from build123d import *

# Parameters (mm, degrees)
SKETCH_1_R              = 67.5
SKETCH_1_R_2            = 32.5
EXTRUDE_1_DEPTH         = 3
HOLE_WIZARD_M12_1_D     = 10.2
HOLE_WIZARD_M12_1_DEPTH = 5
HOLE_WIZARD_M12_1_TIP   = 3.064389157


with BuildPart() as part:
    # 草图1 → 凸台-拉伸1 (new body)
    with BuildSketch(Plane(origin=(0, 0, 0), x_dir=(1, 0, 0), z_dir=(0, 1, 0))):
        with Locations(Location((0, 0, 0), (0, 0, 270))):
            Circle(SKETCH_1_R)
        with Locations(Location((0, 0, 0), (0, 0, 270))):
            Circle(SKETCH_1_R_2, mode=Mode.SUBTRACT)
    extrude(amount=EXTRUDE_1_DEPTH)

    # M12 螺纹孔的螺纹孔钻头1
    with Locations(Plane(origin=(0, 3, 0), x_dir=(1, 0, 0), z_dir=(0, 1, 0))):
        with Locations((0, 55), (-47.631397208, 27.5), (-47.631397208, -27.5), (0, -55), (47.631397208, -27.5), (47.631397208, 27.5)):
            Hole(HOLE_WIZARD_M12_1_D / 2, depth=HOLE_WIZARD_M12_1_DEPTH)
            with Locations((0, 0, -(HOLE_WIZARD_M12_1_DEPTH + HOLE_WIZARD_M12_1_TIP / 2))):  # 118° drill point
                Cone(0, HOLE_WIZARD_M12_1_D / 2, HOLE_WIZARD_M12_1_TIP, mode=Mode.SUBTRACT)


solid = part.part
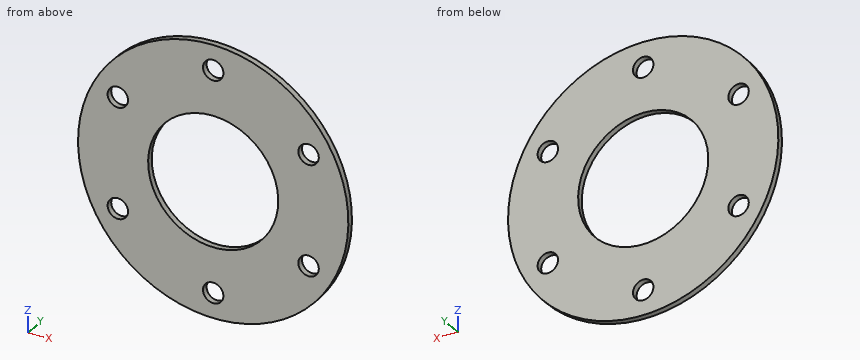
Input: part model. Units: mm. Frame: model coordinates. Coordinates: 2 decimals unless noted, no trailing zeros. Order: outer loops, then holes, each group sorted by start corner. A loop starts at its lowest first (then second) coordinate and runs counter-clockwise, first axis right, second up. Notation, with made-up numbers: M 81.5,-38 L 135.5,-38 A33 ccw 135.5,-9 Z; hole C 27.25,25 d1. An arc over 180 degrees is marked long. Answer in a Markdown table with one row per item.
(1) Material intervals for line 1 (Z direction, x = 52, y = 0.65); line 2 (X direction, y = 0.75, z = 0); line 3 (X direction, y = 1.45, z = -27.5), sorted ascending. Write a range as [from, to].
Numbers:
| item | result |
|---|---|
| line 1 | z = [-43.04, -30.13], [-24.87, 24.87], [30.13, 43.04] |
| line 2 | x = [-67.5, -32.5], [32.5, 67.5] |
| line 3 | x = [-61.64, -52.73], [-42.53, -17.32], [17.32, 42.53], [52.73, 61.64] |
(2) Section query C-C, the plane z = -27.5. Output: boundary loops of the cut face in (x, y).
Numbers:
| item | result |
|---|---|
| outline | M -61.64,0 L -52.73,0 L -52.73,3 L -61.64,3 Z; M -42.53,0 L -17.32,0 L -17.32,3 L -42.53,3 Z; M 17.32,0 L 42.53,0 L 42.53,3 L 17.32,3 Z; M 52.73,0 L 61.64,0 L 61.64,3 L 52.73,3 Z |
(3) Contact query for flat-ended pins moving along their axis: pin 1 Ø1.5 at (x, y) = (-26, 2.5) entering from +Z; pin 2 Ø1 at (x, y) = (-44, 0.5) entering from +Z. Output: stop coordinate, or through.
Numbers:
| item | result |
|---|---|
| pin 1 | stops at z = 62.6 |
| pin 2 | stops at z = 51.61 |
(4) Section query B-B, the plane x = 0. Output: boundary loops of the cut face in (y, z), plus the area to 3 significant figures.
Numbers:
| item | result |
|---|---|
| outline | M 0,-67.5 L 3,-67.5 L 3,-60.1 L 0,-60.1 Z; M 0,-49.9 L 3,-49.9 L 3,-32.5 L 0,-32.5 Z; M 0,32.5 L 3,32.5 L 3,49.9 L 0,49.9 Z; M 0,60.1 L 3,60.1 L 3,67.5 L 0,67.5 Z |
| area | 149 mm^2 |
(5) Section query A-A, the plane z = 0. Output: boundary loops of the cut face in (x, y), plus the area to 3 significant figures.
Numbers:
| item | result |
|---|---|
| outline | M -67.5,0 L -32.5,0 L -32.5,3 L -67.5,3 Z; M 32.5,0 L 67.5,0 L 67.5,3 L 32.5,3 Z |
| area | 210 mm^2 |
(6) Section query D-D, the plane y = 2.45. Output: boundary loops of the cut face in (x, z), plus the area to 3 significant figures.
Numbers:
| item | result |
|---|---|
| outline | C 0,0 d135; hole C -47.63,-27.5 d10.2; hole C -47.63,27.5 d10.2; hole C 0,0 d65; hole C 0,-55 d10.2; hole C 0,55 d10.2; hole C 47.63,-27.5 d10.2; hole C 47.63,27.5 d10.2 |
| area | 10,500 mm^2 |
